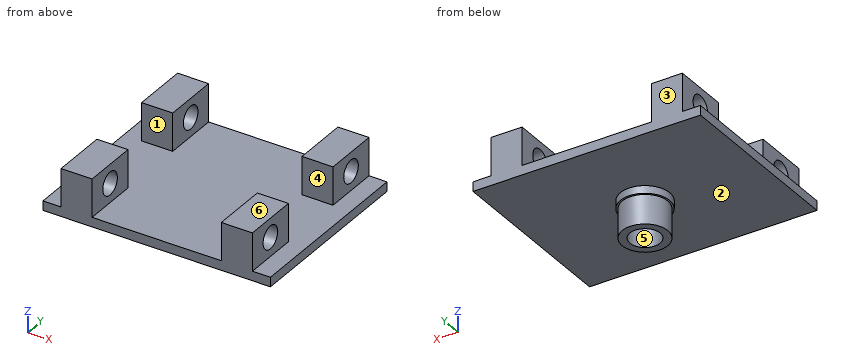
```python
from build123d import *

# Parameters (mm, degrees)
SKETCH1_W           = 600
SKETCH1_H           = 480
BOSS_EXTRUDE1_DEPTH = 25
SKETCH2_W           = 82
SKETCH2_H           = 148
BOSS_EXTRUDE2_DEPTH = 100
SKETCH4_R           = 30
CUT_EXTRUDE1_DEPTH  = 743.483164792
SKETCH5_R           = 65
SKETCH5_R_2         = 40
BOSS_EXTRUDE3_DEPTH = 20
SKETCH6_R           = 60
SKETCH6_R_2         = 40
BOSS_EXTRUDE4_DEPTH = 77
SKETCH7_R           = 40
BOSS_EXTRUDE5_DEPTH = 12.5


with BuildPart() as part:
    # Sketch1 → Boss-Extrude1 (new body)
    with BuildSketch(Plane.XY):
        with Locations((300, 240)):
            Rectangle(SKETCH1_W, SKETCH1_H)
    extrude(amount=BOSS_EXTRUDE1_DEPTH)

    # Sketch2 → Boss-Extrude2 (add)
    with BuildSketch(Plane.XY.offset(25)):
        with Locations((88.5, 406)):
            Rectangle(SKETCH2_W, SKETCH2_H)
        with Locations((88.5, 74)):
            Rectangle(SKETCH2_W, SKETCH2_H)
        with Locations((511.5, 74)):
            Rectangle(SKETCH2_W, SKETCH2_H)
        with Locations((511.5, 406)):
            Rectangle(SKETCH2_W, SKETCH2_H)
    extrude(amount=BOSS_EXTRUDE2_DEPTH)

    # Sketch4 → Cut-Extrude1 (cut, through all)
    with BuildSketch(Plane.ZY.offset(-47.5)):
        with Locations(Location((75, 406, 0), (0, 0, 180))):
            Circle(SKETCH4_R)
        with Locations(Location((75, 74, 0), (0, 0, 180))):
            Circle(SKETCH4_R)
    extrude(amount=-CUT_EXTRUDE1_DEPTH, mode=Mode.SUBTRACT)

    # Sketch5 → Boss-Extrude3 (add)
    with BuildSketch(Plane(origin=(0, 0, 0), x_dir=(-1, 0, 0), z_dir=(0, 0, -1))):
        with Locations((-300, 240)):
            Circle(SKETCH5_R)
        with Locations((-300, 240)):
            Circle(SKETCH5_R_2, mode=Mode.SUBTRACT)
    extrude(amount=BOSS_EXTRUDE3_DEPTH)

    # Sketch6 → Boss-Extrude4 (add)
    with BuildSketch(Plane(origin=(0, 0, -20), x_dir=(-1, 0, 0), z_dir=(0, 0, -1))):
        with Locations((-300, 240)):
            Circle(SKETCH6_R)
        with Locations((-300, 240)):
            Circle(SKETCH6_R_2, mode=Mode.SUBTRACT)
    extrude(amount=BOSS_EXTRUDE4_DEPTH)

    # Sketch7 → Boss-Extrude5 (add)
    with BuildSketch(Plane(origin=(0, 0, 0), x_dir=(-1, 0, 0), z_dir=(0, 0, -1))):
        with Locations((-300, 240)):
            Circle(SKETCH7_R)
    extrude(amount=BOSS_EXTRUDE5_DEPTH)


solid = part.part
```
Verification items for the finished model (mm, model axes). Face numbers are marked on the shaded views. A direction names the side the tool comes from. Coordinates: 2 decimals unless noted, no trailing zeros. Order: outer loops, then holes, each group sorted by start corner. A loop starts at its lowest first (then second) coordinate and runs counter-clockwise, first axis right, second up. Notation, with made-up numbers: (10, 87.25) - (21, 87.25) arc R16 ccw to (21, 107.25) - close; hole circle Ø9 at (10, -16.5). An arc over 180 degrees is marked (long way). Return JSON: item names as keys, results as strings.
(1) Section check A-A, the plane y = 74. Record the cut outline in (x, z), and give its area (3 significant figures).
Filled sheet:
{"outline": "(0, 0) - (600, 0) - (600, 25) - (552.5, 25) - (552.5, 45) - (470.5, 45) - (470.5, 25) - (129.5, 25) - (129.5, 45) - (47.5, 45) - (47.5, 25) - (0, 25) - close; (47.5, 105) - (129.5, 105) - (129.5, 125) - (47.5, 125) - close; (470.5, 105) - (552.5, 105) - (552.5, 125) - (470.5, 125) - close", "area": "21,600 mm^2"}
(2) Section check C-C, the plane z = 34. Record the cut outline in (x, y).
Filled sheet:
{"outline": "(47.5, 0) - (129.5, 0) - (129.5, 148) - (47.5, 148) - close; (47.5, 332) - (129.5, 332) - (129.5, 480) - (47.5, 480) - close; (470.5, 0) - (552.5, 0) - (552.5, 148) - (470.5, 148) - close; (470.5, 332) - (552.5, 332) - (552.5, 480) - (470.5, 480) - close"}
(3) Thickness scan on line 1 along Y through (x, z) = (97, 75); line 2 along Y through (x, z) = (514, 102); line 3 along Z through (x, y) = (503, 406). Record the ranges inside material, lowest first.
Filled sheet:
{"line 1": "y = 0 to 44, 104 to 148, 332 to 376, 436 to 480", "line 2": "y = 0 to 60.92, 87.08 to 148, 332 to 392.92, 419.08 to 480", "line 3": "z = 0 to 45, 105 to 125"}
(4) Section check B-B, the plane x = 59.5. Record the cut outline in (y, z), and give its area (3 significant figures).
Filled sheet:
{"outline": "(0, 0) - (480, 0) - (480, 125) - (332, 125) - (332, 25) - (148, 25) - (148, 125) - (0, 125) - close; hole circle Ø60 at (74, 75); hole circle Ø60 at (406, 75)", "area": "35,900 mm^2"}
(5) Section check D-D, the plane x = 300. Record the cut outline in (y, z).
Filled sheet:
{"outline": "(0, 0) - (175, 0) - (175, -20) - (180, -20) - (180, -97) - (200, -97) - (200, -12.5) - (280, -12.5) - (280, -97) - (300, -97) - (300, -20) - (305, -20) - (305, 0) - (480, 0) - (480, 25) - (0, 25) - close"}
(6) Access from +Z, -Z, +X, -X, +Y, -Y to the whole of each face (thin tool, end or side, straight path). Record for the marked faces 4, 5 and 6.
Filled sheet:
{"face 4": "+Z, +X, -X", "face 5": "-Z", "face 6": "+Z, +X, -X, +Y, -Y"}
(7) Go/stop test with flat-tipped pins: pin 1 (12 mm diameter, centred on x = 528.5, y = 263, fed in from -Z); pin 2 (1.5 mm diameter, centred on y = 96, z = 99.5, fed in from -X). Record where each tip stops, or that it passes through.
Filled sheet:
{"pin 1": "stops at z = 0", "pin 2": "stops at x = 47.5"}
(8) Mould release check, pull along Y, two halves, no side actions. Record for the marked faces 1, 2 and 3: pulls with the +Y half, pulls with the -Y half, needs draft (parallel to the pull), parting line crosses it, or undercut.
Filled sheet:
{"face 1": "undercut", "face 2": "needs draft", "face 3": "pulls with the +Y half"}
